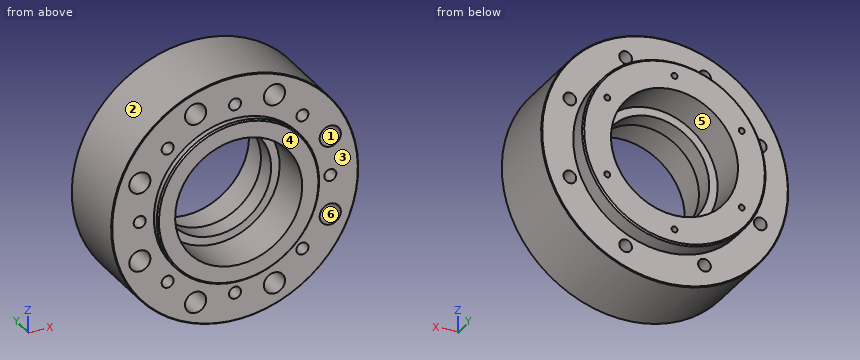
from build123d import *

# Parameters (mm, degrees)
SKETCH1_R                                          = 87.5
BOSS_EXTRUDE1_DEPTH                                = 55
SKETCH2_R                                          = 65
BOSS_EXTRUDE2_DEPTH                                = 13
SKETCH3_R                                          = 57.5
BOSS_EXTRUDE3_DEPTH                                = 5
SKETCH4_R                                          = 45
CUT_EXTRUDE1_DEPTH                                 = 31
CUT_EXTRUDE2_START                                 = -28
SKETCH5_R                                          = 45
CUT_EXTRUDE2_DEPTH                                 = 28
SKETCH6_R                                          = 39
CUT_EXTRUDE3_DEPTH                                 = 132.671940823
CHAMFER1_SIZE                                      = 1
HOLE_SIZE_BASED_ON_SOCKET_HEAD_CAP_SCR_D           = 9
HOLE_SIZE_BASED_ON_SOCKET_HEAD_CAP_SCR_CBORE_D     = 15
HOLE_SIZE_BASED_ON_SOCKET_HEAD_CAP_SCR_CBORE_DEPTH = 30
CIRPATTERN1_COUNT                                  = 8
CHAMFER2_SIZE                                      = 0.5
CIRPATTERN2_COUNT                                  = 8
CIRPATTERN3_COUNT                                  = 6


with BuildPart() as part:
    # Sketch1 → Boss-Extrude1 (new body)
    with BuildSketch(Plane(origin=(0, 0, 0), x_dir=(1, 0, 0), z_dir=(0, 1, 0))):
        with Locations(Location((0, 0, 0), (0, 0, 270))):
            Circle(SKETCH1_R)
    extrude(amount=BOSS_EXTRUDE1_DEPTH)

    # Sketch2 → Boss-Extrude2 (add)
    with BuildSketch(Plane(origin=(0, 55, 0), x_dir=(1, 0, 0), z_dir=(0, 1, 0))):
        with Locations(Location((0, 0, 0), (0, 0, 270))):
            Circle(SKETCH2_R)
    extrude(amount=BOSS_EXTRUDE2_DEPTH)

    # Sketch3 → Boss-Extrude3 (add)
    with BuildSketch(Plane.XZ):
        with Locations(Location((0, 0, 0), (0, 0, 90))):
            Circle(SKETCH3_R)
    extrude(amount=BOSS_EXTRUDE3_DEPTH)

    # Sketch4 → Cut-Extrude1 (cut)
    with BuildSketch(Plane.XZ.offset(5)):
        with Locations(Location((0, 0, 0), (0, 0, 270))):
            Circle(SKETCH4_R)
    extrude(amount=-CUT_EXTRUDE1_DEPTH, mode=Mode.SUBTRACT)

    # Sketch5 → Cut-Extrude2 (cut)
    with BuildSketch(Plane(origin=(0, 68, 0), x_dir=(1, 0, 0), z_dir=(0, 1, 0)).offset(CUT_EXTRUDE2_START)):
        with Locations(Location((0, 0, 0), (0, 0, 90))):
            Circle(SKETCH5_R)
    extrude(amount=CUT_EXTRUDE2_DEPTH, mode=Mode.SUBTRACT)

    # Sketch6 → Cut-Extrude3 (cut, through all)
    with BuildSketch(Plane(origin=(0, 40, 0), x_dir=(1, 0, 0), z_dir=(0, 1, 0))):
        with Locations(Location((0, 0, 0), (0, 0, 270))):
            Circle(SKETCH6_R)
    extrude(amount=-CUT_EXTRUDE3_DEPTH, mode=Mode.SUBTRACT)

    # Chamfer1
    chamfer1_edges = [part.edges().sort_by_distance(p)[0] for p in [
        (0, -5, -57.5),
        (0, 68, -65),
    ]]
    chamfer(chamfer1_edges, length=CHAMFER1_SIZE)

    # Hole size (% based on socket head cap screw type)1 (through all)
    with Locations(Plane(origin=(0, 0, 0), x_dir=(-1, 0, 0), z_dir=(0, -1, 0))):
        with Locations((-67.443205873, 27.935890563)):
            hole_size_based_on_socket_head_cap_scr = CounterBoreHole(HOLE_SIZE_BASED_ON_SOCKET_HEAD_CAP_SCR_D / 2, HOLE_SIZE_BASED_ON_SOCKET_HEAD_CAP_SCR_CBORE_D / 2, HOLE_SIZE_BASED_ON_SOCKET_HEAD_CAP_SCR_CBORE_DEPTH)

    # CirPattern1: Hole size (% based on socket head cap screw type)1 ×8 about axis
    cirpattern1_axis = Axis((0, 0, 0), (0, 1, 0))
    for i in range(1, CIRPATTERN1_COUNT):
        add(hole_size_based_on_socket_head_cap_scr.rotate(cirpattern1_axis, i * 360 / CIRPATTERN1_COUNT), mode=Mode.SUBTRACT)

    # Chamfer2
    chamfer2_edges = [part.edges().sort_by_distance(p)[0] for p in [
        (0, 0, -87.5),
        (0, 55, -87.5),
    ]]
    chamfer(chamfer2_edges, length=CHAMFER2_SIZE)

    # Sketch13 → M10 Tapped Hole1 (revolve, cut)
    with BuildSketch(Plane(origin=(0, 0, -67.5), x_dir=(0, 0, -1), z_dir=(1, 0, 0))):
        Polygon((0, 0), (0, 40.053657631), (4.25, 37.5), (4.25, 0), align=None)
    m10_tapped_hole1 = revolve(axis=Axis((0, -6.35, -67.5), (0, 1, 0)), mode=Mode.SUBTRACT)

    # CirPattern2: M10 Tapped Hole1 ×8 about axis
    cirpattern2_axis = Axis((0, 0, 0), (0, 1, 0))
    for i in range(1, CIRPATTERN2_COUNT):
        add(m10_tapped_hole1.rotate(cirpattern2_axis, i * 360 / CIRPATTERN2_COUNT), mode=Mode.SUBTRACT)

    # Sketch15 → M5 Tapped Hole1 (revolve, cut)
    with BuildSketch(Plane(origin=(0, 68, 55), x_dir=(0, 0, 1), z_dir=(1, 0, 0))):
        Polygon((0, 0), (0, 15.2618073), (2.1, 14), (2.1, 0), align=None)
    m5_tapped_hole1 = revolve(axis=Axis((0, 74.35, 55), (0, -1, 0)), mode=Mode.SUBTRACT)

    # CirPattern3: M5 Tapped Hole1 ×6 about axis
    cirpattern3_axis = Axis((0, 0, 0), (0, 1, 0))
    for i in range(1, CIRPATTERN3_COUNT):
        add(m5_tapped_hole1.rotate(cirpattern3_axis, i * 360 / CIRPATTERN3_COUNT), mode=Mode.SUBTRACT)


solid = part.part
CAD build for the part. Positions are in the model's coordinates, mm. Face numbers are marked on the shaded views. A direction names the side the tool comes from. Round coordinates to 2 decimals unless told otherwise and drop trailing zeros.
(1) Probe line 1 along X through (y, z) = (1, 65.5); line 2 along X through (y, z) = (7, 50); line 3 along X through (y, z) = (61, -27). List the from-to ranges inside material, lowest first.
(2) Drop flat-ended pins along their axis: P1, Ø8, axis at x = 67.44, z = -27.94, coming from the +Y side; P2, Ø2, axis at y = 15.5, z = -5.5, coming from the +X side; P3, Ø7.5, axis at x = 0, z = 67.5, coming from the -Y side; P4, Ø12, axis at x = 12, y = 40.5, coming from the +Z side. Give the stop position or say it passes through.
(3) Mould opens along Z. For the marked faces 1, 2 and 3 say: pulls with the +Z half, pulls with the -Z half, needs draft (parallel to the pull), parting line crosses it, or undercut.
(4) 3-axis set-ups, long thin cutter, end or side, ignore diameter. For the marked faces 4, 5 and 6: which of +Z, -Z, +X, -X, +Y, -Y reach the whole face in a straight line?
From the geometry:
1. line 1: x = -58.02 to -35.18, -20.69 to -3.75, 3.75 to 20.69, 35.18 to 58.02
1. line 2: x = -71.81 to -51.32, -44.14 to 44.14, 51.32 to 71.81
1. line 3: x = -59.13 to -49.67, -45.59 to -36, 36 to 45.59, 49.67 to 59.13
2. P1: passes through
2. P2: stops at x = 87.38
2. P3: stops at y = 37.8
2. P4: stops at z = 87.29
3. face 1: undercut
3. face 2: parting line crosses it
3. face 3: needs draft
4. face 4: +Z, -Z, +X, -X, -Y
4. face 5: +Y
4. face 6: -Y
